Design review of the part built by this model. Coordinates are the model's own, in mm. Face numbers are marked on the shaded views. A direction names the side the tool comes from. Give positions to 0.01 mm unless a question says otherwise; leave off trailing zeros. Loops run counter-clockwise (first coordinate to the right, second up) from the corner with the lowest first, then second, coordinate; pieces in that order, holes last. Notation, with made-up numbers: (81.25, -15) - (130.25, -15) arc R20 cw to (130.25, 4) - close; hole circle Ø1 at (52, 48). An arc over 180 degrees is marked (long way). Write each question's results on one line, items separated by ' | '.
```python
from build123d import *

# Parameters (mm, degrees)
SKETCH1_W                  = 25
SKETCH1_H                  = 17.5
BOSS_EXTRUDE1_DEPTH        = 8
SKETCH2_W                  = 7.5
SKETCH2_H                  = 7
CUT_EXTRUDE1_DEPTH         = 8
SKETCH3_W                  = 9.5
SKETCH3_H                  = 7
CUT_EXTRUDE2_DEPTH         = 18.228247154
SKETCH4_R                  = 2.75
CUT_EXTRUDE3_DEPTH         = 5
F_3_5_3_5_DIAMETER_HOLE1_D = 3.5
CHAMFER1_SIZE              = 1


with BuildPart() as part:
    # Sketch1 → Boss-Extrude1 (new body)
    with BuildSketch(Plane.XY):
        Rectangle(SKETCH1_W, SKETCH1_H)
    extrude(amount=BOSS_EXTRUDE1_DEPTH)

    # Sketch2 → Cut-Extrude1 (cut)
    with BuildSketch(Plane.XY.offset(8)):
        with Locations((8.75, 5.25)):
            Rectangle(SKETCH2_W, SKETCH2_H)
        with Locations((-8.75, 5.25)):
            Rectangle(SKETCH2_W, SKETCH2_H)
    extrude(amount=-CUT_EXTRUDE1_DEPTH, mode=Mode.SUBTRACT)

    # Sketch3 → Cut-Extrude2 (cut, through all)
    with BuildSketch(Plane.XY.offset(8)):
        with Locations((0, -5.25)):
            Rectangle(SKETCH3_W, SKETCH3_H)
    extrude(amount=-CUT_EXTRUDE2_DEPTH, mode=Mode.SUBTRACT)

    # Sketch4 → Cut-Extrude3 (cut)
    with BuildSketch(Plane.XY.offset(8)):
        with Locations((0, 5.25)):
            Circle(SKETCH4_R)
    extrude(amount=-CUT_EXTRUDE3_DEPTH, mode=Mode.SUBTRACT)

    # Ø3.5 (3.5) Diameter Hole1 (through all)
    with Locations(Plane(origin=(0, 1.75, 0), x_dir=(1, 0, 0), z_dir=(0, 1, 0))):
        with Locations((-8.5, -4), (8.5, -4)):
            Hole(F_3_5_3_5_DIAMETER_HOLE1_D / 2)

    # Chamfer1
    chamfer1_edges = [part.edges().sort_by_distance(p)[0] for p in [
        (-12.5, -3.5, 0),
        (-12.5, -3.5, 8),
        (-5, 8.75, 4),
        (5, 8.75, 4),
        (12.5, -3.5, 8),
        (12.5, -3.5, 0),
    ]]
    chamfer(chamfer1_edges, length=CHAMFER1_SIZE)


solid = part.part
```
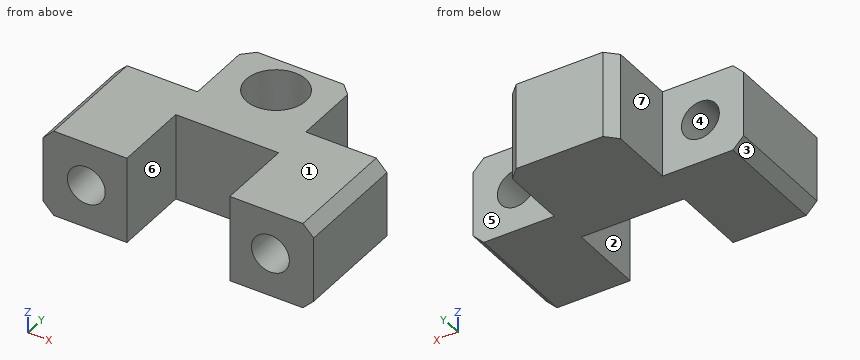
Item 1: Tool access review of the marked faces 5, 6 and 7: name each direction out of +Z, -Z, +X, -X, +Y, -Y from which nothing blocks a thin tool from reaching the whole face with its end or side.
Output values:
face 5: +Z, -Z, +X, +Y | face 6: +Z, -Z, -Y | face 7: +Z, -Z, -X, +Y
Item 2: We need section A-A on y = -7. Give the boundary of the cut face in (x, z), then the cut area to 3 significant figures.
Output values:
outline: (-12.5, 1) - (-11.5, 0) - (-4.75, 0) - (-4.75, 8) - (-11.5, 8) - (-12.5, 7) - close; (4.75, 0) - (11.5, 0) - (12.5, 1) - (12.5, 7) - (11.5, 8) - (4.75, 8) - close; hole circle Ø3.5 at (-8.5, 4); hole circle Ø3.5 at (8.5, 4) | area: 103 mm²
Item 3: Draft analysis for pull direction Z (two halves, no side actions). For the marked faces 1, 2, 3 and 4, state which applies: +Z half, -Z half, draft (parallel to the pull), parting line (faces both ways), or undercut.
Output values:
face 1: +Z half | face 2: draft | face 3: -Z half | face 4: undercut
Item 4: Wall thickness on probe 1 along X at (y, z) = (-2, 4); probe 2 along X at (y, z) = (-8, 6.75); probe 3 along X at (y, z) = (-6.75, 5.25): over which ranges is each line inside the solid? List them lowest first.
Output values:
probe 1: x = -12.5 to -10.25, -6.75 to -4.75, 4.75 to 6.75, 10.25 to 12.5 | probe 2: x = -12.5 to -4.75, 4.75 to 12.5 | probe 3: x = -12.5 to -9.72, -7.28 to -4.75, 4.75 to 7.28, 9.72 to 12.5
Item 5: Clearance check with flat-ended pins moving along their axes: P1, Ø1.8, axis at y = 5, z = 5.5, coming from the +X side; P2, Ø2.5, axis at x = -0.5, z = 5, coming from the -Y side; P3, Ø1.6, axis at x = 1, y = 4, coming from the +Z side; P4, Ø1, axis at x = -9, y = 4, coming from the +Z side. State where each tip first meets the part, or that it passes through.
Output values:
P1: stops at x = 5 | P2: stops at y = -1.75 | P3: stops at z = 3 | P4: passes through
Item 6: We need section D-D on y = 0. Give the boundary of the cut face in (x, z).
Output values:
outline: (-12.5, 1) - (-11.5, 0) - (11.5, 0) - (12.5, 1) - (12.5, 7) - (11.5, 8) - (-11.5, 8) - (-12.5, 7) - close; hole circle Ø3.5 at (-8.5, 4); hole circle Ø3.5 at (8.5, 4)
Item 7: We need section C-C on z = 4.5. Give the boundary of the cut face in (x, y).
Output values:
outline: (-12.5, -8.75) - (-10.18, -8.75) - (-10.18, 1.75) - (-12.5, 1.75) - close; (-6.82, -8.75) - (-4.75, -8.75) - (-4.75, -1.75) - (4.75, -1.75) - (4.75, -8.75) - (6.82, -8.75) - (6.82, 1.75) - (5, 1.75) - (5, 7.75) - (4, 8.75) - (-4, 8.75) - (-5, 7.75) - (-5, 1.75) - (-6.82, 1.75) - close; (10.18, -8.75) - (12.5, -8.75) - (12.5, 1.75) - (10.18, 1.75) - close; hole circle Ø5.5 at (0, 5.25)
Item 8: We need section B-B on x = 8.5. Give the boundary of the cut face in (y, z).
Output values:
outline: (-8.75, 0) - (1.75, 0) - (1.75, 2.25) - (-8.75, 2.25) - close; (-8.75, 5.75) - (1.75, 5.75) - (1.75, 8) - (-8.75, 8) - close
